```python
from build123d import *


with BuildPart() as part:
    # 草图1 → 旋转1 (revolve)
    with BuildSketch(Plane.XY, mode=Mode.PRIVATE) as revolve_1_sk:
        Polygon((-360, 60), (360, 60), (360, 25), (372, 25), (372, 17.5), (451, 17.5), (451, 0), (-451, 0), (-451, 17.5), (-372, 17.5), (-372, 25), (-360, 25), align=None)
    revolve(revolve_1_sk.sketch.rotate(Axis((-451, 0, 0), (1, 0, 0)), 90), axis=Axis((-451, 0, 0), (1, 0, 0)))


solid = part.part
```
The model under review builds one solid part; all positions refer to its coordinate system, in mm. A direction names the side the tool comes from. Round coordinates to 2 decimals unless told otherwise and drop trailing zeros. Order: outer loops, then holes, each group sorted by start corner. A loop starts at its lowest first (then second) coordinate and runs counter-clockwise, first axis right, second up.
Item 1: Machinability: for faces 1 (the flat face through (360, 26, -1)), 2 (the flat face through (451, 0, 0)), 3 (the flat face through (-372, 5, 17)), which of the approach directions +Z, -Z, +X, -X, +Y, -Y give a long, thin tool a straight path to every point of the face, cutting with its end or side? Answer none if there is none.
Working result:
face 1: +X
face 2: +Z, -Z, +X, +Y, -Y
face 3: -X
Item 2: Add section D-D, the plane y = 37. State the section outline as (x, z) points.
Working result:
outline: (-360, -47.23) - (360, -47.23) - (360, 47.23) - (-360, 47.23) - close
Item 3: For pin 1 (8 mm diameter, centred on x = 277.5, y = 27, fed in from +Z); pin 2 (10 mm diameter, centred on x = -192, y = 21, fed in from +Z); pin 3 (6 mm diameter, centred on x = 198.5, y = 11, fed in from +Z), all flat-tipped, find the tip position at first contact; note any pin that passes through.
Working result:
pin 1: stops at z = 55.42
pin 2: stops at z = 57.83
pin 3: stops at z = 59.46
Item 4: Add section A-A, the plane z = 0. State the section outline as (x, y) points.
Working result:
outline: (-451, -17.5) - (-372, -17.5) - (-372, -25) - (-360, -25) - (-360, -60) - (360, -60) - (360, -25) - (372, -25) - (372, -17.5) - (451, -17.5) - (451, 17.5) - (372, 17.5) - (372, 25) - (360, 25) - (360, 60) - (-360, 60) - (-360, 25) - (-372, 25) - (-372, 17.5) - (-451, 17.5) - close
Item 5: Add section C-C, the plane x = -166.5. State the section outline as (y, z) points, and give its area (3 significant figures).
Working result:
outline: circle Ø120 at (0, 0)
area: 11,300 mm2
Item 6: To check wall thickness, follow probe 1 along X at (y, z) = (-46, -13); probe 2 along Y at (x, z) = (89.5, 4.5); probe 3 along Y at (x, z) = (-400.5, -0.5). State the ranges of each line that lie inside material, in increasing order.
Working result:
probe 1: x = -360 to 360
probe 2: y = -59.83 to 59.83
probe 3: y = -17.49 to 17.49
